Geometry check sheet. Reference: the model listing, model coordinates, mm. Face numbers are marked on the shaded views. A direction names the side the tool comes from. Coordinates: 2 decimals unless noted, no trailing zeros. Write each loop counter-clockwise with the first axis right and the second up, starting at its lowest first coordinate (ties: lowest second). Pieces come first, ordered by that corner, then holes. Notation, with made-up numbers: (10.25, 27.5) -> (53.25, 27.5) arc R23 cw to (53.25, 65.5) -> close; hole circle Ø5 at (41.25, 16). An arc over 180 degrees is marked (long way). Use a Markdown table: item, result.
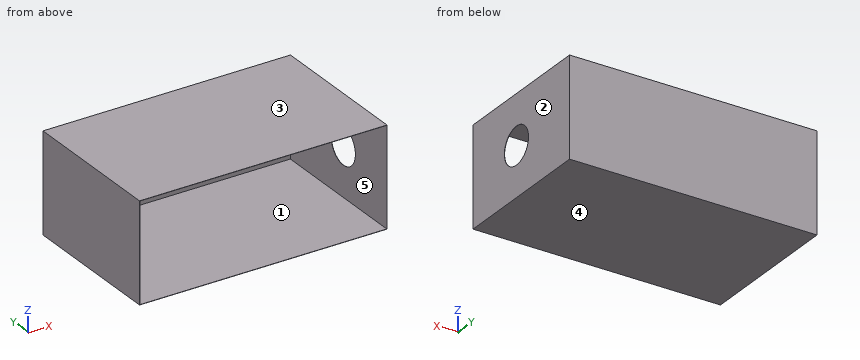
```python
from build123d import *

# Parameters (mm, degrees)
SKETCH1_W           = 1000
SKETCH1_H           = 400
BOSS_EXTRUDE1_DEPTH = 600
SKETCH2_W           = 998
SKETCH2_H           = 398
CUT_EXTRUDE1_DEPTH  = 599
SKETCH3_R           = 75
CUT_EXTRUDE2_DEPTH  = 50


with BuildPart() as part:
    # Sketch1 → Boss-Extrude1 (new body)
    with BuildSketch(Plane(origin=(0, 0, 0), x_dir=(1, 0, 0), z_dir=(0, 1, 0))):
        Rectangle(SKETCH1_W, SKETCH1_H)
    extrude(amount=BOSS_EXTRUDE1_DEPTH)

    # Sketch2 → Cut-Extrude1 (cut)
    with BuildSketch(Plane.XZ):
        Rectangle(SKETCH2_W, SKETCH2_H)
    extrude(amount=-CUT_EXTRUDE1_DEPTH, mode=Mode.SUBTRACT)

    # Sketch3 → Cut-Extrude2 (cut)
    with BuildSketch(Plane(origin=(500, 0, 0), x_dir=(0, 0, -1), z_dir=(1, 0, 0))):
        with Locations((0, 270)):
            Circle(SKETCH3_R)
    extrude(amount=-CUT_EXTRUDE2_DEPTH, mode=Mode.SUBTRACT)


solid = part.part
```
Item 1: Section check C-C on x = 361. Record the boundary of the cut face in (y, z).
Answer block:
| item | result |
|---|---|
| outline | (0, -200) -> (600, -200) -> (600, 200) -> (0, 200) -> (0, 199) -> (599, 199) -> (599, -199) -> (0, -199) -> close |
Item 2: Thickness scan on L1, parallel to X at y = 558, z = 165; L2, parallel to Z at x = 341.5, y = 122.5; L3, parallel to Y at x = 499.5, z = 0. Record the ranges inside material, lowest first. Write a range as [from, to].
Answer block:
| item | result |
|---|---|
| L1 | x = [-500, -499], [499, 500] |
| L2 | z = [-200, -199], [199, 200] |
| L3 | y = [0, 195], [345, 600] |
Item 3: Section check D-D on z = 169.5. Record the boundary of the cut face in (x, y), then the cut area to 3 significant figures.
Answer block:
| item | result |
|---|---|
| outline | (-500, 0) -> (-499, 0) -> (-499, 599) -> (499, 599) -> (499, 0) -> (500, 0) -> (500, 600) -> (-500, 600) -> close |
| area | 2,200 mm^2 |
Item 4: Section check A-A on z = 0. Record the boundary of the cut face in (x, y), then the cut area to 3 significant figures.
Answer block:
| item | result |
|---|---|
| outline | (-500, 0) -> (-499, 0) -> (-499, 599) -> (499, 599) -> (499, 345) -> (500, 345) -> (500, 600) -> (-500, 600) -> close; (499, 0) -> (500, 0) -> (500, 195) -> (499, 195) -> close |
| area | 2,050 mm^2 |
Item 5: Mould release check, pull along Z, two halves, no side actions. Record for the marked faces 1, 2 and 3: +Z half, -Z half, draft (parallel to the pull), parting line (faces both ways), or undercut.
Answer block:
| item | result |
|---|---|
| face 1 | undercut |
| face 2 | draft |
| face 3 | +Z half |
Item 6: Section check B-B on y = 455. Record the boundary of the cut face in (x, z).
Answer block:
| item | result |
|---|---|
| outline | (-500, -200) -> (500, -200) -> (500, 200) -> (-500, 200) -> close; hole (-499, -199) -> (499, -199) -> (499, 199) -> (-499, 199) -> close |
Item 7: Tool access check on the marked faces 4 and 5. Record the directions out of +Z, -Z, +X, -X, +Y, -Y that give a thin tool (end or side, any length) a straight path to the whole face; none if there is none.
Answer block:
| item | result |
|---|---|
| face 4 | -Z, +X, -X, +Y, -Y |
| face 5 | -Y |
